```python
from build123d import *

# Parameters (mm, degrees)
SKETCH_2_R             = 12.5
EXTRUDE_1_DEPTH        = 304.5
SKETCH_3_OUTSIDE_W     = 149.006
SKETCH_3_OUTSIDE_H     = 149.006
SKETCH_3_OUTSIDE_R     = 8.5
CUT_EXTRUDE_1_DEPTH    = 173.5
CUT_EXTRUDE_2_DEPTH    = 3
CUT_EXTRUDE_3_DEPTH    = 4
CHAMFER_1_SIZE         = 0.5
CHAMFER_2_SIZE         = 0.3
SKETCH_8_W             = 1.2
SKETCH_8_H             = 0.55
PATTERN_LINEAR_2_COUNT = 2
PATTERN_LINEAR_2_PITCH = 34.2
SKETCH_9_W             = 1.1
SKETCH_9_H             = 0.4
PATTERN_LINEAR_3_COUNT = 2
PATTERN_LINEAR_3_PITCH = 34.1
FILLET_1_R             = 1.5


with BuildPart() as part:
    # 草图2 → 凸台-拉伸1 (new, symmetric)
    with BuildSketch(Plane(origin=(0, 0, 0), x_dir=(0, 0, -1), z_dir=(1, 0, 0))):
        Circle(SKETCH_2_R)
    extrude(amount=EXTRUDE_1_DEPTH, both=True)

    # 草图3 outside → 切除-拉伸1 (cut)
    with BuildSketch(Plane.ZY.offset(304.5)):
        Rectangle(SKETCH_3_OUTSIDE_W, SKETCH_3_OUTSIDE_H)
        Circle(SKETCH_3_OUTSIDE_R, mode=Mode.SUBTRACT)
    extrude(amount=-CUT_EXTRUDE_1_DEPTH, mode=Mode.SUBTRACT)

    # 草图5 → 切除-拉伸2 (cut)
    with BuildSketch(Plane.XY.offset(8.5)):
        with BuildLine():
            Line((-267.5, 2.5), (-242.5, 2.5))
            ThreePointArc((-242.5, 2.5), (-240, 0), (-242.5, -2.5))
            Line((-242.5, -2.5), (-267.5, -2.5))
            ThreePointArc((-267.5, -2.5), (-270, 0), (-267.5, 2.5))
        make_face()
        with BuildLine():
            Line((-217.5, 2.5), (-147.5, 2.5))
            ThreePointArc((-147.5, 2.5), (-145, 0), (-147.5, -2.5))
            Line((-147.5, -2.5), (-217.5, -2.5))
            ThreePointArc((-217.5, -2.5), (-220, 0), (-217.5, 2.5))
        make_face()
    extrude(amount=-CUT_EXTRUDE_2_DEPTH, mode=Mode.SUBTRACT)

    # 草图6 → 切除-拉伸3 (cut)
    with BuildSketch(Plane.XY.offset(12.5)):
        with BuildLine():
            Line((238.5, 4), (258.5, 4))
            ThreePointArc((258.5, 4), (262.5, 0), (258.5, -4))
            Line((258.5, -4), (238.5, -4))
            ThreePointArc((238.5, -4), (234.5, 0), (238.5, 4))
        make_face()
    extrude(amount=-CUT_EXTRUDE_3_DEPTH, mode=Mode.SUBTRACT)

    # 倒角1
    chamfer_1_edges = [part.edges().sort_by_distance(p)[0] for p in [
        (304.5, 0, 12.5),
        (-131, 0, 12.5),
    ]]
    chamfer(chamfer_1_edges, length=CHAMFER_1_SIZE)

    # 倒角2
    chamfer_2_edges = [part.edges().sort_by_distance(p)[0] for p in [
        (-304.5, 0, -8.5),
    ]]
    chamfer(chamfer_2_edges, length=CHAMFER_2_SIZE)

    # 草图8 → 切除-旋转2 (revolve, cut)
    with BuildSketch(Plane.XY, mode=Mode.PRIVATE) as cut_revolve_2_sk:
        with Locations((267.1, -12.225)):
            Rectangle(SKETCH_8_W, SKETCH_8_H)
    cut_revolve_2 = revolve(cut_revolve_2_sk.sketch.rotate(Axis((304.5, 0, 0), (-1, 0, 0)), 90), axis=Axis((304.5, 0, 0), (-1, 0, 0)), mode=Mode.SUBTRACT)

    # 阵列(线性)2: 切除-旋转2 ×2
    with Locations(*[(-i * PATTERN_LINEAR_2_PITCH, 0, 0) for i in range(1, PATTERN_LINEAR_2_COUNT)]):
        add(cut_revolve_2, mode=Mode.SUBTRACT)

    # 草图9 → 切除-旋转3 (revolve, cut)
    with BuildSketch(Plane.XY, mode=Mode.PRIVATE) as cut_revolve_3_sk:
        with Locations((-272.05, -8.3)):
            Rectangle(SKETCH_9_W, SKETCH_9_H)
    cut_revolve_3 = revolve(cut_revolve_3_sk.sketch.rotate(Axis((-131, 0, 0), (-1, 0, 0)), 270), axis=Axis((-131, 0, 0), (-1, 0, 0)), mode=Mode.SUBTRACT)

    # 阵列(线性)3: 切除-旋转3 ×2
    with Locations(*[(i * PATTERN_LINEAR_3_PITCH, 0, 0) for i in range(1, PATTERN_LINEAR_3_COUNT)]):
        add(cut_revolve_3, mode=Mode.SUBTRACT)

    # 圆角1
    fillet_1_edges = [part.edges().sort_by_distance(p)[0] for p in [
        (-131, 0, -8.5),
    ]]
    fillet(fillet_1_edges, radius=FILLET_1_R)


solid = part.part
```
Could you check a few things on this model? Use its own coordinates, in mm. A direction names the side the tool comes from. Round coordinates to 2 decimals unless told otherwise and drop trailing zeros. Loops run counter-clockwise (first coordinate to the right, second up) from the corner with the lowest first, then second, coordinate; pieces in that order, holes last.
Q1. I want a section at A-A (x = 171). Write out the boundary of the cut face in (y, z).
Q2. On a 3-axis mill with a long thin cutter (end or side, diameter ignored), from which of +Z, -Z, +X, -X, +Y, -Y can I reach the whole of each face in a straight line? I mean faces 1 (the cylindrical face through (267.11, 10.08, 6.42)), 2 (the cylindrical face through (-288.621, 7.167, 4.57)), 3 (the cylindrical face through (250.231, 3.755, -11.923)). Say none if no direction works.
Q3. Please list where these lines run through material, in increasing order: L1, parallel to Z at x = -5, y = -4; L2, parallel to X at y = -5.75, z = -9.5; L3, parallel to Z at x = -57.5, y = 9.25.
Q4. Thinking about a two-plate mould opening in X: for faces 4 (the cylindrical face through (-185.684, 7.167, 4.57)), 5 (the cylindrical face through (-237.942, 4.929, 6.428)), 6 (the flat face through (-131, 9, -5)), which applies, pulls with the +X half, pulls with the -X half, needs draft (parallel to the pull), parting line crosses it, or undercut?
Q5. For P1, Ø5, axis at x = -23, y = 9.5, coming from the -Z side; P2, Ø1.3, axis at x = -258, z = 7, coming from the -Y side; P3, Ø1.5, axis at x = -199.5, y = -1, coming from the +Z side, each with a flat end and sliding along its axis, tell me the tip position at first contact or that it passes through.
Q6. I want a section at B-B (x = -155.5). Write out the boundary of the cut face in (y, z), and give its area (3 significant figures).
Answer below:
1. outline: circle Ø25 at (0, 0)
2. face 1: none
2. face 2: -X
2. face 3: +X, -X
3. L1: z = -11.84 to 11.84
3. L2: x = -131 to 304.5
3. L3: z = -8.41 to 8.41
4. face 4: needs draft
4. face 5: undercut
4. face 6: pulls with the -X half
5. P1: stops at z = -10.36
5. P2: stops at y = -5.65
5. P3: stops at z = 5.5
6. outline: (-2.5, 5.5) - (-2.5, 8.12) arc R8.5 ccw (long way) to (2.5, 8.12) - (2.5, 5.5) - close
6. area: 213 mm2
